from build123d import *

# Parameters (mm, degrees)
KEYWAY_SKETCH_W  = 20
KEYWAY_SKETCH_H  = 5
KEYWAY_CUT_DEPTH = 3


with BuildPart() as part:
    # Shaft Profile Sketch → Stepped Shaft Body (revolve)
    with BuildSketch(Plane.XY, mode=Mode.PRIVATE) as stepped_shaft_body_sk:
        Polygon((0, 0), (0, 9.5), (7, 9.5), (7, 6.5), (13, 6.5), (13, 9.5), (20, 9.5), (20, 12.5), (30, 12.5), (30, 10), (130, 10), (130, 0), align=None)
    revolve(stepped_shaft_body_sk.sketch.rotate(Axis((0, 0, 0), (1, 0, 0)), 90), axis=Axis((0, 0, 0), (1, 0, 0)))

    # Keyway Sketch → Keyway Cut (cut, symmetric)
    with BuildSketch(Plane.XY):
        with Locations((120, 9.5)):
            Rectangle(KEYWAY_SKETCH_W, KEYWAY_SKETCH_H)
    extrude(amount=KEYWAY_CUT_DEPTH, both=True, mode=Mode.SUBTRACT)


solid = part.part
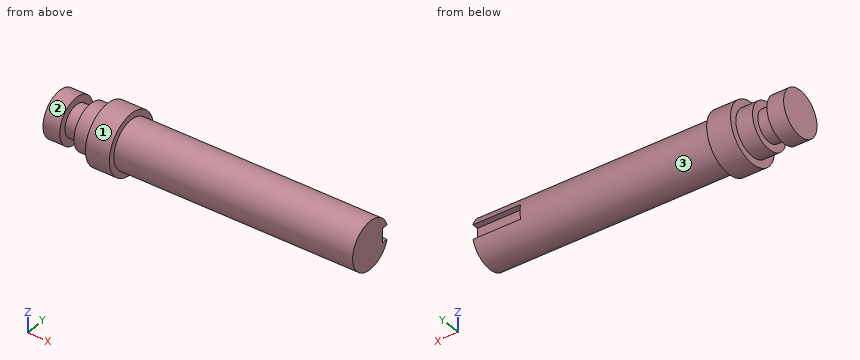
Read the model definition and answer for the solid it produces. Units are mm, in the model's axes. Face numbers are marked on the shaded views. A direction names the side the tool comes from. Round coordinates to 2 decimals unless told otherwise and drop trailing zeros. Write each loop counter-clockwise with the first axis right and the second up, starting at its lowest first coordinate (ties: lowest second). Pieces come first, ordered by that corner, then holes. Notation, with made-up numbers: (-15.75, 53) - (0.25, 53) arc R20 cw to (0.25, 84) - close; hole circle Ø6 at (-33.5, 79.25). An arc over 180 degrees is marked (long way). One line per question, with ' | ' between items. Start each with the question number.
1. Section D-D (x = 22) is taken. Determine the outline of the cut face in (y, z), and give its area (3 significant figures).
2. For the marked faces 1, 2 and 3, determine the directions among +Z, -Z, +X, -X, +Y, -Y from which every point of the face is accessible in a straight line to the end or side of a thin tool.
3. Section A-A (y = 0) is taken. Determine the outline of the cut face in (x, z), and give its area (3 significant figures).
4. Section B-B (z = 0) is taken. Determine the outline of the cut face in (x, y), and give its area (3 significant figures).
5. Each of these flat-tipped pins is pushed along its axis until it touches: pin 1 (12 mm diameter, centred on x = 113.5, z = 2.5, fed in from +Y); pin 2 (0.8 mm diameter, centred on x = 119, y = 9, fed in from -Z); pin 3 (5 mm diameter, centred on x = 43, z = 0.5, fed in from -Y). Where does it stop, or does it pass through?
6. Find the intervals of material crossed by probe 1 along X at (y, z) = (8.5, 5.5); probe 2 along X at (y, z) = (-2.75, -8); probe 3 along Z at (x, y) = (98.5, 0.5), in increasing order. Write a range as [from, to].
7. Section C-C (x = 112.5) is taken. Determine the outline of the cut face in (y, z), and give its area (3 significant figures).
Filled in:
1) outline: circle Ø25 at (0, 0) | area: 491 mm²
2) face 1: +X, -X | face 2: -X | face 3: +X
3) outline: (0, -9.5) - (7, -9.5) - (7, -6.5) - (13, -6.5) - (13, -9.5) - (20, -9.5) - (20, -12.5) - (30, -12.5) - (30, -10) - (130, -10) - (130, 10) - (30, 10) - (30, 12.5) - (20, 12.5) - (20, 9.5) - (13, 9.5) - (13, 6.5) - (7, 6.5) - (7, 9.5) - (0, 9.5) - close | area: 2,590 mm²
4) outline: (0, -9.5) - (7, -9.5) - (7, -6.5) - (13, -6.5) - (13, -9.5) - (20, -9.5) - (20, -12.5) - (30, -12.5) - (30, -10) - (130, -10) - (130, 7) - (110, 7) - (110, 10) - (30, 10) - (30, 12.5) - (20, 12.5) - (20, 9.5) - (13, 9.5) - (13, 6.5) - (7, 6.5) - (7, 9.5) - (0, 9.5) - close | area: 2,530 mm²
5) pin 1: y = 10 | pin 2: z = -5.1 | pin 3: y = -10
6) probe 1: [20, 30] | probe 2: [0, 7], [13, 130] | probe 3: [-9.99, 9.99]
7) outline: (7, -3) - (7, 3) - (9.54, 3) arc R10 ccw (long way) to (9.54, -3) - close | area: 297 mm²
